Work out the finished part from the listing and answer in its coordinate system (mm). A direction names the side the tool comes from. Round coordinates to 2 decimals unless told otherwise and drop trailing zeros. Order: outer loops, then holes, each group sorted by start corner. A loop starts at its lowest first (then second) coordinate and runs counter-clockwise, first axis right, second up. Notation, with made-up numbers: (46.25, 75) - (94.25, 75) arc R20 cw to (94.25, 106) - close; hole circle Ø1 at (-6, 57). An arc over 180 degrees is marked (long way). Use CSV: the item, a comma, the result in double quotes.
from build123d import *

# Parameters (mm, degrees)
SKETCH_1_W             = 150
SKETCH_1_H             = 25
BOSS_EXTRUDE_1_DEPTH   = 18
SKETCH_2_W             = 16
SKETCH_2_H             = 23
CUT_EXTRUDE_1_DEPTH    = 152.592381075
CUT_EXTRUDE_3_DEPTH    = 79.136099212
F_4_5_4_5_HOLE_1_D     = 4.5
F_4_5_4_5_HOLE_1_DEPTH = 15
F_4_5_4_5_HOLE_1_TIP   = 1.351936393
F_4_5_4_5_HOLE_3_D     = 4.5
F_4_5_4_5_HOLE_3_DEPTH = 15
F_4_5_4_5_HOLE_3_TIP   = 1.351936393
F_4_5_4_5_HOLE_2_D     = 4.5
F_4_5_4_5_HOLE_2_DEPTH = 15
F_4_5_4_5_HOLE_2_TIP   = 1.351936393
CHAMFER_1_SIZE         = 2
FILLET_1_R             = 2
SKETCH_11_W            = 150
SKETCH_11_H            = 2
CUT_EXTRUDE_4_DEPTH    = 10
CHAMFER_4_SIZE         = 5
SKETCH_12_W            = 121.932032981
SKETCH_12_H            = 48.36827262
CUT_EXTRUDE_5_DEPTH    = 78.699742599
CHAMFER_5_SIZE         = 5
SKETCH_13_W            = 80
SKETCH_13_H            = 2
CUT_EXTRUDE_6_DEPTH    = 10


with BuildPart() as part:
    # Sketch 1 → Boss-Extrude 1 (new body)
    with BuildSketch(Plane(origin=(0, 0, 0), x_dir=(-1, 0, 0), z_dir=(0, 0, -1))):
        Rectangle(SKETCH_1_W, SKETCH_1_H)
    extrude(amount=-BOSS_EXTRUDE_1_DEPTH)

    # Sketch 2 → Cut-Extrude 1 (cut, through all)
    with BuildSketch(Plane.ZY.offset(75)):
        with Locations((8, -1)):
            Rectangle(SKETCH_2_W, SKETCH_2_H)
    extrude(amount=-CUT_EXTRUDE_1_DEPTH, mode=Mode.SUBTRACT)

    # Sketch 4 → Cut-Extrude 3 (cut, through all)
    with BuildSketch(Plane.XY.offset(18)):
        with BuildLine():
            Line((-69, -6.25), (-4, -6.25))
            ThreePointArc((-4, -6.25), (-1.25, -3.5), (-4, -0.75))
            Line((-4, -0.75), (-69, -0.75))
            ThreePointArc((-69, -0.75), (-71.75, -3.5), (-69, -6.25))
        make_face()
    extrude(amount=-CUT_EXTRUDE_3_DEPTH, mode=Mode.SUBTRACT)

    # Ø4.5 (4.5) Hole 1
    with Locations(Plane(origin=(0, 12.5, 0), x_dir=(-1, 0, 0), z_dir=(0, 1, 0))):
        with Locations((-60, 8)):
            Hole(F_4_5_4_5_HOLE_1_D / 2, depth=F_4_5_4_5_HOLE_1_DEPTH)
            with Locations((0, 0, -(F_4_5_4_5_HOLE_1_DEPTH + F_4_5_4_5_HOLE_1_TIP / 2))):  # 118° drill point
                Cone(0, F_4_5_4_5_HOLE_1_D / 2, F_4_5_4_5_HOLE_1_TIP, mode=Mode.SUBTRACT)

    # Ø4.5 (4.5) Hole 3
    with Locations(Plane(origin=(0, 12.5, 0), x_dir=(-1, 0, 0), z_dir=(0, 1, 0))):
        with Locations((60, 8)):
            Hole(F_4_5_4_5_HOLE_3_D / 2, depth=F_4_5_4_5_HOLE_3_DEPTH)
            with Locations((0, 0, -(F_4_5_4_5_HOLE_3_DEPTH + F_4_5_4_5_HOLE_3_TIP / 2))):  # 118° drill point
                Cone(0, F_4_5_4_5_HOLE_3_D / 2, F_4_5_4_5_HOLE_3_TIP, mode=Mode.SUBTRACT)

    # Ø4.5 (4.5) Hole 2
    with Locations(Plane(origin=(0, 12.5, 0), x_dir=(-1, 0, 0), z_dir=(0, 1, 0))):
        with Locations((10, 8)):
            Hole(F_4_5_4_5_HOLE_2_D / 2, depth=F_4_5_4_5_HOLE_2_DEPTH)
            with Locations((0, 0, -(F_4_5_4_5_HOLE_2_DEPTH + F_4_5_4_5_HOLE_2_TIP / 2))):  # 118° drill point
                Cone(0, F_4_5_4_5_HOLE_2_D / 2, F_4_5_4_5_HOLE_2_TIP, mode=Mode.SUBTRACT)

    # Chamfer 1
    chamfer_1_edges = [part.edges().sort_by_distance(p)[0] for p in [
        (75, -12.5, 17),
    ]]
    chamfer(chamfer_1_edges, length=CHAMFER_1_SIZE)

    # Fillet 1
    fillet_1_edges = [part.edges().sort_by_distance(p)[0] for p in [
        (0, 12.5, 18),
    ]]
    fillet(fillet_1_edges, radius=FILLET_1_R)

    # Sketch 11 → Cut-Extrude 4 (cut)
    with BuildSketch(Plane(origin=(0, 12.5, 0), x_dir=(1, 0, 0), z_dir=(0, 1, 0))):
        with Locations((0, -1)):
            Rectangle(SKETCH_11_W, SKETCH_11_H)
    extrude(amount=-CUT_EXTRUDE_4_DEPTH, mode=Mode.SUBTRACT)

    # Chamfer 4
    chamfer_4_edges = [part.edges().sort_by_distance(p)[0] for p in [
        (75, 11.5, 2),
        (-75, 11.5, 2),
    ]]
    chamfer(chamfer_4_edges, length=CHAMFER_4_SIZE)

    # Sketch 12 → Cut-Extrude 5 (cut, through all)
    with BuildSketch(Plane(origin=(0, 0, 2), x_dir=(-1, 0, 0), z_dir=(0, 0, -1))):
        with Locations((-65.966016491, 1.254835332)):
            Rectangle(SKETCH_12_W, SKETCH_12_H)
    extrude(amount=-CUT_EXTRUDE_5_DEPTH, mode=Mode.SUBTRACT)

    # Chamfer 5
    chamfer_5_edges = [part.edges().sort_by_distance(p)[0] for p in [
        (5, 11.5, 2),
    ]]
    chamfer(chamfer_5_edges, length=CHAMFER_5_SIZE)

    # Sketch 13 → Cut-Extrude 6 (cut)
    with BuildSketch(Plane(origin=(0, 0, 16), x_dir=(-1, 0, 0), z_dir=(0, 0, -1))):
        with Locations((35, -11.5)):
            Rectangle(SKETCH_13_W, SKETCH_13_H)
    extrude(amount=-CUT_EXTRUDE_6_DEPTH, mode=Mode.SUBTRACT)


solid = part.part
(1) For faces 1 (the cylindrical face through (-1.25, -3.56, 17.01)), 2 (the flat face through (2, 11, 4)), 3 (the flat face through (-36, 0, 16)), determine the directions among +Z, -Z, +X, -X, +Y, -Y from which every point of the face is accessible in a straight line to the end or side of a thin tool.
Findings below:
face 1,"+Z, -Z"
face 2,"-Z, +X, +Y, -Y"
face 3,"-Z, +X, -X, -Y"
(2) Find section B-B (z = 8). Determine the outline of the cut face in (x, y), and give its area (3 significant figures).
Findings below:
outline,"(-75, 10.5) - (-62.25, 10.5) - (-62.25, 12.5) - (-75, 12.5) - close; (-57.75, 10.5) - (-12.25, 10.5) - (-12.25, 12.5) - (-57.75, 12.5) - close; (-7.75, 10.5) - (5, 10.5) - (5, 12.5) - (-7.75, 12.5) - close"
area,"142 mm²"
(3) Each of these flat-tipped pins is pushed along its axis until it touches: pin 1 (5 mm diameter, centred on x = -37, y = -6, fed in from -Z); pin 2 (2 mm diameter, centred on x = -33.5, z = 17, fed in from +Y); pin 3 (1 mm diameter, centred on y = -1.5, z = 14.5, fed in from -X); pin 4 (2 mm diameter, centred on x = -26, z = 13.5, fed in from -Y). Where does it stop, or does it pass through?
Findings below:
pin 1,"stops at z = 16"
pin 2,"stops at y = 12.5"
pin 3,"passes through"
pin 4,"stops at y = 10.5"
(4) Find section A-A (x = -10). Determine the outline of the cut face in (y, z), and give its area (3 significant figures).
Findings below:
outline,"(-10.5, 16) - (-6.25, 16) - (-6.25, 18) - (-10.5, 18) - close; (-0.75, 16) - (10.5, 16) - (10.5, 10.25) - (12.5, 10.25) - (12.5, 16) arc R2 ccw to (10.5, 18) - (-0.75, 18) - close; (10.5, 2) - (12.5, 2) - (12.5, 5.75) - (10.5, 5.75) - close"
area,"53.1 mm²"
(5) Find section D-D (z = 16.75). Determine the outline of the cut face in (x, y), and give its area (3 significant figures).
Findings below:
outline,"(-75, -10.5) - (5, -10.5) - (5, 12.35) - (-75, 12.35) - close; hole (-69, -6.25) - (-4, -6.25) arc R2.75 ccw to (-4, -0.75) - (-69, -0.75) arc R2.75 ccw to start"
area,"1,450 mm²"
(6) The mould has two halves that part along Z. Classify faces 4 (the flat face through (-35, 12, 2)), 5 (the cylindrical face through (-11.66, 11.49, 9.52)), 6 (the flat face through (-36, 10.5, 9)): released by +Z, released by -Z, zero draft, split by the parting line, or undercut.
Findings below:
face 4,"released by -Z"
face 5,"undercut"
face 6,"zero draft"
(7) Find the intervals of material crossed by L1, parallel to Y at x = -50, z = 3.75; L2, parallel to Z at x = -71, y = 5.75; L3, parallel to Z at x = -60, y = 11.5, in increasing order. Write a range as from..to.
Findings below:
L1,"y = 10.5..12.5"
L2,"z = 16..18"
L3,"z = 2..5.75, 10.25..17.73"
(8) Find section C-C (x = -55). Determine the outline of the cut face in (y, z).
Findings below:
outline,"(-10.5, 16) - (-6.25, 16) - (-6.25, 18) - (-10.5, 18) - close; (-0.75, 16) - (10.5, 16) - (10.5, 2) - (12.5, 2) - (12.5, 16) arc R2 ccw to (10.5, 18) - (-0.75, 18) - close"
